The model under review builds one solid part; all positions refer to its coordinate system, in mm. A direction names the side the tool comes from. Coordinates: 2 decimals unless noted, no trailing zeros. Loops run counter-clockwise (first coordinate to the right, second up) from the corner with the lowest first, then second, coordinate; pieces in that order, holes last. Notation, with made-up numbers: M 28.25,57 L 39.25,57 A28 cw 39.25,95 Z; hole C 7.5,-16 d3. An arc over 180 degrees is marked long. Return JSON: item names as keys, results as strings.
```python
from build123d import *

# Parameters (mm, degrees)
BASE_DEPTH = 50


with BuildPart() as part:
    # Sketch1 → Base (new body)
    with BuildSketch(Plane.YZ):
        with BuildLine():
            Line((0, 40), (0, 0))
            Line((0, 0), (40, 0))
            Line((40, 0), (40, 2.666666667))
            ThreePointArc((40, 2.666666667), (39.609475708, 3.609475708), (38.666666667, 4))
            Line((38.666666667, 4), (9, 4))
            ThreePointArc((9, 4), (5.464466094, 5.464466094), (4, 9))
            Line((4, 9), (4, 38.666666667))
            ThreePointArc((4, 38.666666667), (3.609475708, 39.609475708), (2.666666667, 40))
            Line((2.666666667, 40), (0, 40))
        make_face()
    extrude(amount=BASE_DEPTH)


solid = part.part
```
1. Add section B-B on z = 6. Give the boundary of the cut face in (x, y).
Check values:
{"outline": "M 0,0 L 50,0 L 50,5 L 0,5 Z"}
2. Insertion check: pin 1 Ø2 at (x, z) = (36.5, 4) entering from -Y; pin 2 Ø9 at (x, y) = (27.5, 25.5) entering from +Z; pin 3 Ø3 at (x, z) = (19, 6.5) entering from +Y; pin 4 Ø2 at (x, z) = (39, 24) entering from +Y. Each pin has a flat end and moves straight along its axis. Give the tip position at first contact, or say it passes through.
Check values:
{"pin 1": "y = 0", "pin 2": "z = 4", "pin 3": "y = 6", "pin 4": "y = 4"}
3. Machinability: for faces 1 (the face through (25, 1, 40)), 2 (the face through (25, 4, 24)), which of the approach directions +Z, -Z, +X, -X, +Y, -Y give a long, thin tool a straight path to every point of the face, cutting with its end or side? Answer none if there is none.
Check values:
{"face 1": "+Z, +X, -X, +Y, -Y", "face 2": "+Z, +X, -X, +Y"}
4. To check wall thickness, follow line 1 (Z direction, x = 32.5, y = 20); line 2 (Z direction, x = 28.5, y = 3). State the ranges of each line that lie inside material, in increasing order.
Check values:
{"line 1": "0 to 4", "line 2": "0 to 39.96"}
5. Add section A-A on x = 41.5. Give the boundary of the cut face in (y, z).
Check values:
{"outline": "M 0,0 L 40,0 L 40,2.67 A1.33 ccw 38.67,4 L 9,4 A5 cw 4,9 L 4,38.67 A1.33 ccw 2.67,40 L 0,40 Z"}
6. Add section C-C on y = 24. Give the boundary of the cut face in (x, z).
Check values:
{"outline": "M 0,0 L 50,0 L 50,4 L 0,4 Z"}
